from build123d import *

# Parameters (mm, degrees)
SKETCH_1_W          = 80
SKETCH_1_H          = 21
EXTRUDE_1_DEPTH     = 8
SKETCH_2_W          = 80
SKETCH_2_H          = 3
EXTRUDE_2_DEPTH     = 4
CUT_EXTRUDE_1_DEPTH = 8


with BuildPart() as part:
    # 草图1 → 凸台-拉伸1 (new body)
    with BuildSketch(Plane.XY):
        with Locations((0, 10.5)):
            Rectangle(SKETCH_1_W, SKETCH_1_H)
    extrude(amount=EXTRUDE_1_DEPTH)

    # 草图2 → 凸台-拉伸2 (add)
    with BuildSketch(Plane.XY.offset(8)):
        with Locations((0, 1.5)):
            Rectangle(SKETCH_2_W, SKETCH_2_H)
    extrude(amount=EXTRUDE_2_DEPTH)

    # 草图3 → 切除-拉伸1 (cut)
    with BuildSketch(Plane.XY.offset(8)):
        with BuildLine():
            Line((-22.25, 17), (-22.25, 11))
            ThreePointArc((-22.25, 11), (-25, 8.25), (-27.75, 11))
            Line((-27.75, 11), (-27.75, 17))
            ThreePointArc((-27.75, 17), (-25, 19.75), (-22.25, 17))
        make_face()
    cut_extrude_1 = extrude(amount=-CUT_EXTRUDE_1_DEPTH, mode=Mode.SUBTRACT)

    # 镜向1: 切除-拉伸1 across plane
    add(cut_extrude_1.mirror(Plane.ZY), mode=Mode.SUBTRACT)


solid = part.part
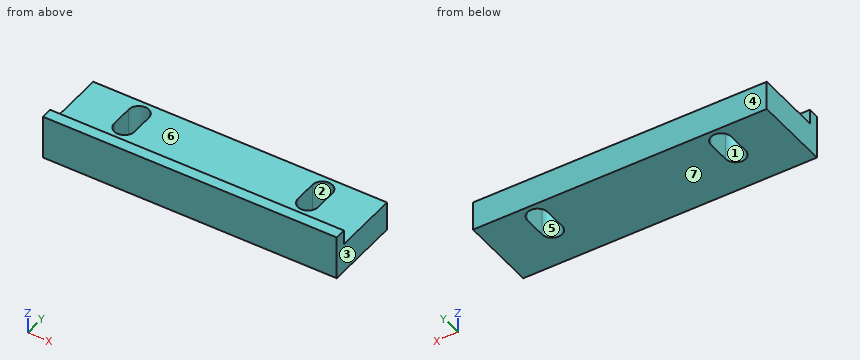
The listing builds one solid part. Answer for the finished solid, in the listing's coordinates (mm). Face numbers are marked on the shaded views. A direction names the side the tool comes from. Round coordinates to 2 decimals unless told otherwise and drop trailing zeros. Write each loop counter-clockwise with the first axis right and the second up, starting at its lowest first coordinate (ties: lowest second). Pieces come first, ordered by that corner, then holes. Notation, with made-up numbers: M 69,5 L 105,5 A25 cw 105,31 Z; hole C -27,38.25 d8. An arc over 180 degrees is marked long. Write each question's results on one line, items separated by ' | '. Start each with the question number.
Item 1: Flat-ended cylindrical pins translate along their axes: pin 1 Ø6 at (x, y) = (-26.5, 11) entering from +Z; pin 2 Ø1.5 at (x, y) = (24, 2.5) entering from -Z. Find the tip coordinate at first contact, or state that the pin passes through.
Item 2: A cutting plane is placed at D-D on y = 9.25. Write down the section's boundary in (x, z).
Item 3: A cutting plane is placed at A-A on y = 13. Write down the section's boundary in (x, z).
Item 4: Straight lines are drawn through the part: L1, parallel to X at y = 14.75, z = 5; L2, parallel to X at y = 10, z = 2.75; L3, parallel to Z at x = 5.5, y = 16.25. For each, find the intervals that lie inside material, in ascending order. Write a range as [from, to].
Item 5: A cutting plane is placed at B-B on x = 25. Write down the section's boundary in (y, z), and give its area (3 significant figures).
Item 6: For the marked faces 5, 6 and 7, determine the directions among +Z, -Z, +X, -X, +Y, -Y from which every point of the face is accessible in a straight line to the end or side of a thin tool.
Item 7: For a pull along X with two mould halves and no side action, classify the marked faces 1, 2, 3 and 4 as pulls with the +X half, pulls with the -X half, needs draft (parallel to the pull), parting line crosses it, or undercut.
Item 8: A cutting plane is placed at C-C on z = 6.5. Write down the section's boundary in (x, y).
Check sheet entries:
1) pin 1: z = 8 | pin 2: z = 0
2) outline: M -40,0 L -27.12,0 L -27.12,8 L -40,8 Z; M -22.88,0 L 22.88,0 L 22.88,8 L -22.88,8 Z; M 27.12,0 L 40,0 L 40,8 L 27.12,8 Z
3) outline: M -40,0 L -27.75,0 L -27.75,8 L -40,8 Z; M -22.25,0 L 22.25,0 L 22.25,8 L -22.25,8 Z; M 27.75,0 L 40,0 L 40,8 L 27.75,8 Z
4) L1: [-40, -27.75], [-22.25, 22.25], [27.75, 40] | L2: [-40, -27.56], [-22.44, 22.44], [27.56, 40] | L3: [0, 8]
5) outline: M 0,0 L 8.25,0 L 8.25,8 L 3,8 L 3,12 L 0,12 Z; M 19.75,0 L 21,0 L 21,8 L 19.75,8 Z | area: 88.0 mm²
6) face 5: +Z, -Z | face 6: +Z, +X, -X, +Y | face 7: -Z, +X, -X, +Y, -Y
7) face 1: undercut | face 2: undercut | face 3: pulls with the +X half | face 4: needs draft
8) outline: M -40,0 L 40,0 L 40,21 L -40,21 Z; hole M -27.75,11 A2.75 ccw -22.25,11 L -22.25,17 A2.75 ccw -27.75,17 Z; hole M 22.25,11 A2.75 ccw 27.75,11 L 27.75,17 A2.75 ccw 22.25,17 Z
